Model file for the job. Use its own axes, mm. A direction names the side the tool comes from. Coordinates: 2 decimals unless noted, no trailing zeros. Write each loop counter-clockwise with the first axis right and the second up, starting at its lowest first coordinate (ties: lowest second). Pieces come first, ordered by that corner, then holes. Notation, with made-up numbers: M 27.25,81 L 33.25,81 A19 cw 33.25,95 Z; hole C 74.5,10.25 d1. An arc over 180 degrees is marked long. One line per question, with ' | ' between items. Start each with the question number.
(1) Cut at A-A (z = 19.5). Write the cut outline in (x, y), plus the area to 3 significant figures.
(2) Two-plate mould, pull along X, no slides. Class faces 1 (the face through (-2.4, -0.1, 40)), 2 (the face through (2.06, 1.58, 35.91)), 3 (the face through (-2.075, 0.013, 39.113)), 4 (the face through (2.47, -1.44, 39.11)): +X half, -X half, draft (parallel to the pull), parting line (faces both ways), or undercut.
(3) Flat gauge pins, fed straight in: pin 1 Ø1.2 at (x, y) = (1.5, -2.5) entering from -Z; pin 2 Ø6 at (y, z) = (3, 9) entering from -X; pin 3 Ø5 at (y, z) = (4.5, 23.5) entering from -X; pin 4 Ø2 at (x, y) = (4, 4.5) entering from -Z. Where does each tip first touch, or does it go through?
(4) Tool access for faces 5 (the face through (-1.05, -1.79, 39.11)), 6 (the face through (1.2, 2.1, 38.2)): list every direction of +Z, -Z, +X, -X, +Y, -Y with a clear straight run to the whole face (end or side of a thin tool).
(5) Wall check: probe 1 along X at (y, z) = (1.5, 2); probe 2 along Z at (x, y) = (-1.75, -2.5); probe 3 along Y at (x, z) = (-0.5, 25). Give the ranges that are in metal, low to high.
from build123d import *

# Parameters (mm, degrees)
SKETCH1_R          = 3
BASE_EXTRUDE_DEPTH = 34.7
CUT_EXTRUDE1_DEPTH = 1.8


with BuildPart() as part:
    # Sketch1 → Base-Extrude (new body)
    with BuildSketch(Plane.XY):
        Circle(SKETCH1_R)
    extrude(amount=BASE_EXTRUDE_DEPTH)

    # Sketch6 → Base-Revolve2 (revolve)
    with BuildSketch(Plane(origin=(0, 0, 0), x_dir=(1, 0, 0), z_dir=(0, 1, 0)), mode=Mode.PRIVATE) as base_revolve2_sk:
        Polygon((2.598, -36.7), (5.65, -39.752), (5.65, -40), (0, -40), (0, -34.7), (3, -34.7), (2.598, -35.102), align=None)
    revolve(base_revolve2_sk.sketch.rotate(Axis((0, 0, -0.393620135), (0, 0, 1)), 180), axis=Axis((0, 0, -0.393620135), (0, 0, 1)))

    # Sketch7 → Cut-Extrude1 (cut)
    with BuildSketch(Plane.XY.offset(40)):
        with BuildLine():
            ThreePointArc((0.489815827, 2.817743859), (0, 2.86), (-0.489815827, 2.817743859))
            ThreePointArc((-0.489815827, 2.817743859), (-0.617632508, 2.737888703), (-0.653418206, 2.591487427))
            ThreePointArc((-0.653418206, 2.591487427), (-1.0375, 1.797002713), (-1.917584843, 1.861620479))
            ThreePointArc((-1.917584843, 1.861620479), (-2.062264916, 1.903829794), (-2.19532985, 1.833064879))
            ThreePointArc((-2.19532985, 1.833064879), (-2.476832655, 1.43), (-2.685145677, 0.984678981))
            ThreePointArc((-2.685145677, 0.984678981), (-2.679897424, 0.83405891), (-2.571003048, 0.729866948))
            ThreePointArc((-2.571003048, 0.729866948), (-2.075, 0), (-2.571003048, -0.729866948))
            ThreePointArc((-2.571003048, -0.729866948), (-2.679897424, -0.83405891), (-2.685145677, -0.984678981))
            ThreePointArc((-2.685145677, -0.984678981), (-2.476832655, -1.43), (-2.19532985, -1.833064879))
            ThreePointArc((-2.19532985, -1.833064879), (-2.062264916, -1.903829794), (-1.917584843, -1.861620479))
            ThreePointArc((-1.917584843, -1.861620479), (-1.0375, -1.797002713), (-0.653418206, -2.591487427))
            ThreePointArc((-0.653418206, -2.591487427), (-0.617632508, -2.737888703), (-0.489815827, -2.817743859))
            ThreePointArc((-0.489815827, -2.817743859), (0, -2.86), (0.489815827, -2.817743859))
            ThreePointArc((0.489815827, -2.817743859), (0.617632508, -2.737888703), (0.653418206, -2.591487427))
            ThreePointArc((0.653418206, -2.591487427), (1.0375, -1.797002713), (1.917584843, -1.861620479))
            ThreePointArc((1.917584843, -1.861620479), (2.062264916, -1.903829794), (2.19532985, -1.833064879))
            ThreePointArc((2.19532985, -1.833064879), (2.476832655, -1.43), (2.685145677, -0.984678981))
            ThreePointArc((2.685145677, -0.984678981), (2.679897424, -0.83405891), (2.571003048, -0.729866948))
            ThreePointArc((2.571003048, -0.729866948), (2.075, 0), (2.571003048, 0.729866948))
            ThreePointArc((2.571003048, 0.729866948), (2.679897424, 0.83405891), (2.685145677, 0.984678981))
            ThreePointArc((2.685145677, 0.984678981), (2.476832655, 1.43), (2.19532985, 1.833064879))
            ThreePointArc((2.19532985, 1.833064879), (2.062264916, 1.903829794), (1.917584843, 1.861620479))
            ThreePointArc((1.917584843, 1.861620479), (1.0375, 1.797002713), (0.653418206, 2.591487427))
            ThreePointArc((0.653418206, 2.591487427), (0.617632508, 2.737888703), (0.489815827, 2.817743859))
        make_face()
    extrude(amount=-CUT_EXTRUDE1_DEPTH, mode=Mode.SUBTRACT)

    # Sketch8 → 切除－旋转1 (revolve, cut)
    with BuildSketch(Plane(origin=(0, 0, 0), x_dir=(1, 0, 0), z_dir=(0, 1, 0))):
        Polygon((0, -38.2), (2.86, -38.2), (0, -37.15904513), align=None)
    revolve(axis=Axis((0, 0, 0), (0, 0, 1)), mode=Mode.SUBTRACT)


solid = part.part
Filled in:
1) outline: C 0,0 d6 | area: 28.3 mm²
2) face 1: draft | face 2: parting line | face 3: undercut | face 4: undercut
3) pin 1: z = 0 | pin 2: x = -3 | pin 3: x = -2.24 | pin 4: z = 39.12
4) face 5: +Z | face 6: none
5) probe 1: -2.6 to 2.6 | probe 2: 37.15 to 40 | probe 3: -2.96 to 2.96
